The model under review builds one solid part; all positions refer to its coordinate system, in mm. Round coordinates to 2 decimals unless told otherwise and drop trailing zeros. Write each loop counter-clockwise with the first axis right and the second up, starting at its lowest first coordinate (ties: lowest second). Pieces come first, ordered by that corner, then holes. Notation, with made-up numbers: M -34,53.5 L 9,53.5 A22 ccw 9,73.5 Z; hole C 20.25,-1.5 d5. An arc over 180 degrees is marked long. Write item = value, one per line. Start each with the question number.
Item 1: Take a section at A-A, the plane x = -14. Give the boundary of the cut face in (y, z), plus the area to 3 significant figures.
Item 2: Take a section at B-B, the plane z = 2. Give the boundary of the cut face in (x, y), plus the area to 3 significant figures.
Item 3: To check wall thickness, follow line 1 along Y through (x, z) = (-23.7, 4.25); line 2 along X through (y, z) = (-71, 5); line 3 along Y through (x, z) = (-9.85, 6.5). State the ranges of each line that lie inside material, in increasing order.
Item 4: For pin 1 Ø1.5 at (x, y) = (9.85, 21.1) entering from +Z; pin 2 Ø3 at (x, z) = (20, 5) entering from -Y; pin 3 Ø14.5 at (x, y) = (0, 45) entering from +Z, all flat-tipped, find the tip position at first contact; note any pin that passes through.
from build123d import *

# Parameters (mm, degrees)
SKETCH1_W             = 60
SKETCH1_H             = 150
BOSS_EXTRUDE1_DEPTH   = 10
CHAMFER1_SIZE         = 5
SKETCH2_R             = 11
CUT_EXTRUDE1_DEPTH    = 6
SKETCH3_R             = 5.5
CUT_EXTRUDE2_DEPTH    = 82
M4_TAPPED_HOLE1_D     = 3.3
M4_TAPPED_HOLE2_D     = 3.3
M4_TAPPED_HOLE2_DEPTH = 11.5
M4_TAPPED_HOLE2_TIP   = 0.991420021
M3_TAPPED_HOLE1_D     = 2.5


with BuildPart() as part:
    # Sketch1 → Boss-Extrude1 (new body)
    with BuildSketch(Plane.XY):
        Rectangle(SKETCH1_W, SKETCH1_H)
    extrude(amount=BOSS_EXTRUDE1_DEPTH)

    # Chamfer1
    chamfer1_edges = [part.edges().sort_by_distance(p)[0] for p in [
        (-30, 75, 5),
        (30, 75, 5),
    ]]
    chamfer(chamfer1_edges, length=CHAMFER1_SIZE)

    # Sketch2 → Cut-Extrude1 (cut)
    with BuildSketch(Plane.XY.offset(10)):
        with Locations((0, 45)):
            Circle(SKETCH2_R)
    extrude(amount=-CUT_EXTRUDE1_DEPTH, mode=Mode.SUBTRACT)

    # Sketch3 → Cut-Extrude2 (cut, through all)
    with BuildSketch(Plane.XY.offset(4)):
        with Locations((0, 45)):
            Circle(SKETCH3_R)
    extrude(amount=-CUT_EXTRUDE2_DEPTH, mode=Mode.SUBTRACT)

    # M4 Tapped Hole1 (through all)
    with Locations(Plane.XY.offset(10)):
        with Locations((-14, 45), (14, 45)):
            Hole(M4_TAPPED_HOLE1_D / 2)

    # M4 Tapped Hole2
    with Locations(Plane(origin=(0, -75, 0), x_dir=(-1, 0, 0), z_dir=(0, -1, 0))):
        with Locations((20, -5), (-20, -5)):
            Hole(M4_TAPPED_HOLE2_D / 2, depth=M4_TAPPED_HOLE2_DEPTH)
            with Locations((0, 0, -(M4_TAPPED_HOLE2_DEPTH + M4_TAPPED_HOLE2_TIP / 2))):  # 118° drill point
                Cone(0, M4_TAPPED_HOLE2_D / 2, M4_TAPPED_HOLE2_TIP, mode=Mode.SUBTRACT)

    # M3 Tapped Hole1 (through all)
    with Locations(Plane(origin=(0, 0, 0), x_dir=(-1, 0, 0), z_dir=(0, 0, -1))):
        with Locations((-9.85, 21.1), (9.85, 21.1), (23.7, 35.95), (23.7, 55.65)):
            Hole(M3_TAPPED_HOLE1_D / 2)


solid = part.part
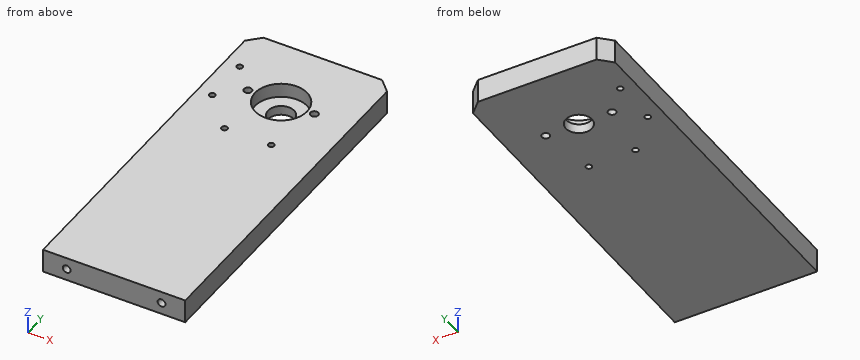
Response values:
q1.outline = M -75,0 L 43.35,0 L 43.35,10 L -75,10 Z; M 46.65,0 L 75,0 L 75,10 L 46.65,10 Z
q1.area = 1,470 mm2
q2.outline = M -30,-75 L 30,-75 L 30,70 L 25,75 L -25,75 L -30,70 Z; hole C -23.7,35.95 d2.5; hole C -23.7,55.65 d2.5; hole C -14,45 d3.3; hole C -9.85,21.1 d2.5; hole C 0,45 d11; hole C 9.85,21.1 d2.5; hole C 14,45 d3.3
q2.area = 8,840 mm2
q3.line_1 = -75 to 34.7, 37.2 to 54.4, 56.9 to 75
q3.line_2 = -30 to -21.65, -18.35 to 18.35, 21.65 to 30
q3.line_3 = -75 to 19.85, 22.35 to 40.1, 49.9 to 75
q4.pin_1 = through
q4.pin_2 = -63.41
q4.pin_3 = 4
